```python
from build123d import *

# Parameters (mm, degrees)
SHELL1_T = -2.5


with BuildPart() as part:
    # Sketch1 → Revolve1 (revolve)
    with BuildSketch(Plane.XY, mode=Mode.PRIVATE) as revolve1_sk:
        Polygon((0, 0), (0, 300), (25, 300), (25, 280), (50, 260), (55, 0), align=None)
    revolve(revolve1_sk.sketch.rotate(Axis((0, 0, 0), (0, 1, 0)), 90), axis=Axis((0, 0, 0), (0, 1, 0)))

    # Shell1
    shell1_openings = [part.faces().sort_by_distance(p)[0] for p in [
        (0, 300, 0),
        (0, 0, 0),
    ]]
    offset(amount=SHELL1_T, openings=shell1_openings, kind=Kind.INTERSECTION)


solid = part.part
```
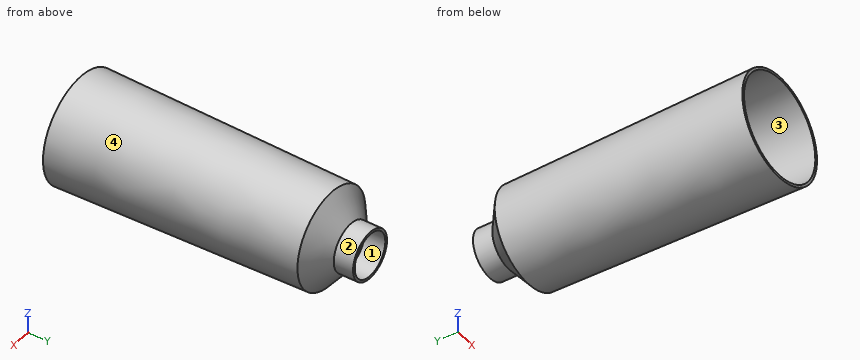
Part model, mm, in its own coordinate system. Face numbers are marked on the shaded views. A direction names the side the tool comes from. Round coordinates to 2 decimals unless told otherwise and drop trailing zeros. Write each loop counter-clockwise with the first axis right and the second up, starting at its lowest first coordinate (ties: lowest second). Pieces come first, ordered by that corner, then holes.
Item 1: Which spindle directions (+Z, -Z, +X, -X, +Y, -Y) get a long thin tool onto all of the face, cutting with end or side? Do the marked faces 1 and 2. Say none if no direction does.
Results:
face 1: +Y, -Y
face 2: +Y
Item 2: Cut at A-A, the plane y = 69. Give the cut face in (x, z).
Results:
outline: circle Ø107.35 at (0, 0); hole circle Ø102.35 at (0, 0)
Item 3: Drop flat-ended pins along their axis: pin 1 Ø12 at (x, z) = (11, 23.5) entering from -Y; pin 2 Ø8 at (x, z) = (-7, 28.5) entering from +Y; pin 3 Ø1 at (x, y) = (9, 85.5) entering from +Z. Give the stop position or say it passes through.
Results:
pin 1: stops at y = 271.24
pin 2: stops at y = 279.72
pin 3: stops at z = 52.67
Item 4: Cut at B-B, the plane y = 140. Give the cut face in (x, z), plus the area to 3 significant figures.
Results:
outline: circle Ø104.62 at (0, 0); hole circle Ø99.61 at (0, 0)
area: 802 mm2
Item 5: Probe L1, parallel to X at y = 290, z = 0; L2, parallel to X at y = 155.5, z = 11; L3, parallel to Z at x = -30.5, y = 214. List the from-to ranges inside material, lowest first.
Results:
L1: x = -25 to -22.5, 22.5 to 25
L2: x = -50.83 to -48.27, 48.27 to 50.83
L3: z = -40.73 to -37.56, 37.56 to 40.73
Item 6: Two-plate mould, pull along Z, no slides. Class the marked faces 3 and 4: +Z half, -Z half, draft (parallel to the pull), parting line (faces both ways), or undercut.
Results:
face 3: undercut
face 4: parting line
